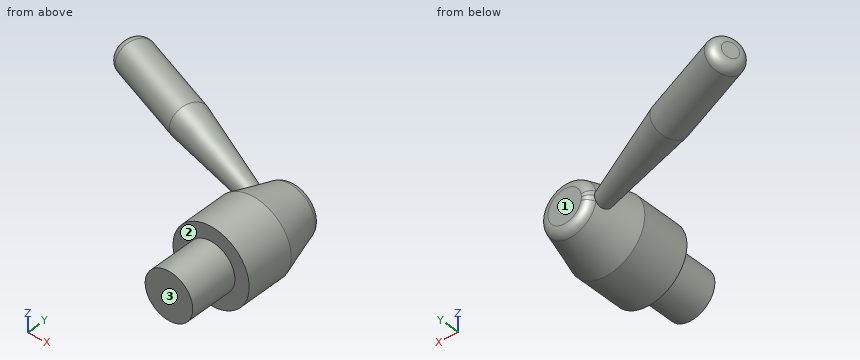
from build123d import *

# Parameters (mm, degrees)
SKETCH4_R           = 5
BOSS_EXTRUDE1_DEPTH = 10
FILLET1_R           = 2


with BuildPart() as part:
    # Sketch2 → Revolve1 (revolve)
    with BuildSketch(Plane.XY):
        Polygon((0, 0), (0, 10), (0, 20), (-5, 20), (-8, 10), (-8, 0), align=None)
    revolve(axis=Axis((0, 20, 0), (0, -1, 0)))

    # Sketch3 → Revolve2 (revolve)
    with BuildSketch(Plane.XY, mode=Mode.PRIVATE) as revolve2_sk:
        Polygon((-45.457291118, 32.007434158), (-46.721063236, 28.616826036), (-27.844496784, 21.581014904), (-4.192388941, 14.958215321), (-3.646298208, 16.423336801), align=None)
    revolve(revolve2_sk.sketch.rotate(Axis((-3.646298208, 16.423336801, 0), (-0.9370274611537507, 0.34925569006639867, 0)), 180), axis=Axis((-3.646298208, 16.423336801, 0), (-0.9370274611537507, 0.34925569006639867, 0)))

    # Sketch4 → Boss-Extrude1 (add)
    with BuildSketch(Plane.XZ):
        Circle(SKETCH4_R)
    extrude(amount=BOSS_EXTRUDE1_DEPTH)

    # Fillet1
    fillet1_edges = [part.edges().sort_by_distance(p)[0] for p in [
        (-46.721063236, 28.616826036, 0),
        (5, 20, 0),
    ]]
    fillet(fillet1_edges, radius=FILLET1_R)


solid = part.part
Verification items for the finished model (mm, model axes). Face numbers are marked on the shaded views. A direction names the side the tool comes from. Coordinates: 2 decimals unless noted, no trailing zeros. Write each loop counter-clockwise with the first axis right and the second up, starting at its lowest first coordinate (ties: lowest second). Pieces come first, ordered by that corner, then holes. Notation, with made-up numbers: M 23,62.5 L 53,62.5 A26 ccw 53,101.5 Z; hole C -31.75,64 d10. An arc over 180 degrees is marked long. Use a Markdown table: item, result.
Q1. Sectioned sample at A-A, the plane y = 12.5. Record the boundary of the cut face in (x, z).
Reply:
| item | result |
|---|---|
| outline | C 0,0 d14.5 |
Q2. Sectioned sample at B-B, the plane y = -6. Record the boundary of the cut face in (x, z), plus the area to 3 significant figures.
Reply:
| item | result |
|---|---|
| outline | C 0,0 d10 |
| area | 78.5 mm² |
Q3. Thickness scan on line 1 (Y direction, x = 0.5, z = -1); line 2 (Z direction, x = -39, y = 30.5); line 3 (X direction, y = 0.5, z = 0). Record the ranges inside material, lowest first.
Reply:
| item | result |
|---|---|
| line 1 | y = -10 to 20 |
| line 2 | z = -3.52 to 3.52 |
| line 3 | x = -8 to 8 |
Q4. Go/stop test with flat-tipped pins: P1, Ø3, axis at y = -5, z = 3.5, coming from the +X side; P2, Ø4, axis at y = 20.5, z = -5.5, coming from the -X side; P3, Ø4, axis at x = -25.5, z = -1, coming from the +Y side; P4, Ø6, axis at y = 0, z = 0.5, coming from the +X side. Record where each tip stops, or that it passes through.
Reply:
| item | result |
|---|---|
| P1 | stops at x = 4.58 |
| P2 | stops at x = -3.21 |
| P3 | stops at y = 29.12 |
| P4 | stops at x = 8 |
Q5. Set-up check for the marked faces 1, 2 and 3: record each of +Z, -Z, +X, -X, +Y, -Y from which the full face is reachable in a straight line by a thin tool's end or side.
Reply:
| item | result |
|---|---|
| face 1 | +Z, -Z, +X, +Y |
| face 2 | -Y |
| face 3 | +Z, -Z, +X, -X, -Y |
